```python
from build123d import *

# Parameters (mm, degrees)
BOSS_EXTRUDE1_DEPTH = 4
SKETCH2_OUTSIDE_W   = 21.324
SKETCH2_OUTSIDE_H   = 19.776
SKETCH2_OUTSIDE_R   = 5
CUT_EXTRUDE1_DEPTH  = 4
CUT_EXTRUDE1_DRAFT  = -30
SKETCH3_R           = 3
BOSS_EXTRUDE2_DEPTH = 16
CHAMFER1_SIZE       = 0.5


with BuildPart() as part:
    # Sketch1 → Boss-Extrude1 (new body)
    with BuildSketch(Plane.XY):
        Polygon((2.886751346, 5), (-2.886751346, 5), (-5.773502692, 0), (-2.886751346, -5), (2.886751346, -5), (5.773502692, 0), align=None)
    extrude(amount=BOSS_EXTRUDE1_DEPTH)


with BuildPart() as cut_extrude1_tool:
    # Sketch2 outside → Cut-Extrude1 (with draft: the straight prism first)
    with BuildSketch(Plane(origin=(0, 0, 0), x_dir=(-1, 0, 0), z_dir=(0, 0, -1))):
        Rectangle(SKETCH2_OUTSIDE_W, SKETCH2_OUTSIDE_H)
        Circle(SKETCH2_OUTSIDE_R, mode=Mode.SUBTRACT)
    extrude(amount=-CUT_EXTRUDE1_DEPTH)
    # Cut-Extrude1: the draft: its side faces are tilted about the plane it starts from
    cut_extrude1_sides = [cut_extrude1_tool.faces().sort_by_distance(p)[0] for p in [
        (0, -9.888, 2),
        (-10.662, 0, 2),
        (0, 9.888, 2),
        (10.662, 0, 2),
        (5, 0, 2),
    ]]
    draft(cut_extrude1_sides, Plane(origin=(0, 0, 0), x_dir=(-1, 0, 0), z_dir=(0, 0, -1)), CUT_EXTRUDE1_DRAFT)


with BuildPart() as part_1:
    add(part.part)

    # Cut-Extrude1: cut by cut_extrude1_tool
    add(cut_extrude1_tool.part, mode=Mode.SUBTRACT)

    # Sketch3 → Boss-Extrude2 (add)
    with BuildSketch(Plane.XY.offset(4)):
        Circle(SKETCH3_R)
    extrude(amount=BOSS_EXTRUDE2_DEPTH)

    # Chamfer1
    chamfer1_edges = [part_1.edges().sort_by_distance(p)[0] for p in [
        (-3, 0, 20),
    ]]
    chamfer(chamfer1_edges, length=CHAMFER1_SIZE)


solid = part_1.part
```
CAD build for the part. Positions are in the model's coordinates, mm. A direction names the side the tool comes from. Coordinates: 2 decimals unless noted, no trailing zeros. Order: outer loops, then holes, each group sorted by start corner. A loop starts at its lowest first (then second) coordinate and runs counter-clockwise, first axis right, second up. Notation, with made-up numbers: M 35.5,-30.5 L 88.5,-30.5 A19 ccw 88.5,-26.5 Z; hole C 84.25,74.25 d9. An arc over 180 degrees is marked long. Write each question's results on one line, items separated by ' | '. Start each with the question number.
Q1. Which spindle directions (+Z, -Z, +X, -X, +Y, -Y) get a long thin tool onto all of the face, cutting with end or side? Do faces 1 (the flat face through (2.5, 2.3, 4)), 2 (the flat face through (4.31, -2.535, 1.972)). Say none if no direction does.
Q2. Cut at A-A (z = 13.5). List the corners of the cut face in (x, y).
Q3. Drill centre lines: probe 1 along Z at (x, y) = (-4.25, -2); probe 2 along X at (y, z) = (-0.5, 7.25); probe 3 along X at (y, z) = (-2.75, 2.5). Where is each one in solid material? Low to high. Write a range as from..to.
Q4. Flat gauge pins, fed straight in: P1, Ø1.5, axis at x = 0, z = 8.5, coming from the -Y side; P2, Ø3, axis at x = -2, y = 0.5, coming from the -Z side; P3, Ø3, axis at x = 3.5, y = 2, coming from the +Z side. Where does each tip first touch, or does it go through?
Found:
1) face 1: +Z | face 2: +Z, -Z, +X, -Y
2) outline: C 0,0 d6
3) probe 1: 0..4 | probe 2: -2.96..2.96 | probe 3: -4.19..4.19
4) P1: y = -3 | P2: z = 0 | P3: z = 19.97
